The model under review builds one solid part; all positions refer to its coordinate system, in mm. Face numbers are marked on the shaded views. A direction names the side the tool comes from. Round coordinates to 2 decimals unless told otherwise and drop trailing zeros. Write each loop counter-clockwise with the first axis right and the second up, starting at its lowest first coordinate (ties: lowest second). Pieces come first, ordered by that corner, then holes. Notation, with made-up numbers: (24.25, 74) - (80.25, 74) arc R17 ccw to (80.25, 82) - close; hole circle Ø7 at (30, 88). An arc over 180 degrees is marked (long way). Write each question's results on one line, items separated by ' | '.
```python
from build123d import *

# Parameters (mm, degrees)
BOSS_EXTRUDE1_DEPTH   = 140
M8_TAPPED_HOLE1_D     = 6.8
M8_TAPPED_HOLE1_DEPTH = 19.75
M8_TAPPED_HOLE1_TIP   = 2.042926105


with BuildPart() as part:
    # Sketch1 → Boss-Extrude1 (new body)
    with BuildSketch(Plane.XY):
        with BuildLine():
            Line((0, 0), (0, 42.5))
            ThreePointArc((0, 42.5), (3.807611845, 51.692388155), (13, 55.5))
            Line((13, 55.5), (103, 55.5))
            ThreePointArc((103, 55.5), (112.192388155, 51.692388155), (116, 42.5))
            Line((116, 42.5), (116, 0))
            Line((116, 0), (108, 0))
            Line((108, 0), (108, 42.5))
            ThreePointArc((108, 42.5), (106.535533906, 46.035533906), (103, 47.5))
            Line((103, 47.5), (13, 47.5))
            ThreePointArc((13, 47.5), (9.464466094, 46.035533906), (8, 42.5))
            Line((8, 42.5), (8, 0))
            Line((8, 0), (0, 0))
        make_face()
    extrude(amount=BOSS_EXTRUDE1_DEPTH)

    # M8 Tapped Hole1
    with Locations(Plane(origin=(0, 55.5, 0), x_dir=(1, 0, 0), z_dir=(0, 1, 0))):
        with Locations((28.5, -13), (87.5, -13), (87.5, -53), (28.5, -53), (28.5, -87), (87.5, -87), (87.5, -127), (28.5, -127)):
            Hole(M8_TAPPED_HOLE1_D / 2, depth=M8_TAPPED_HOLE1_DEPTH)
            with Locations((0, 0, -(M8_TAPPED_HOLE1_DEPTH + M8_TAPPED_HOLE1_TIP / 2))):  # 118° drill point
                Cone(0, M8_TAPPED_HOLE1_D / 2, M8_TAPPED_HOLE1_TIP, mode=Mode.SUBTRACT)


solid = part.part
```
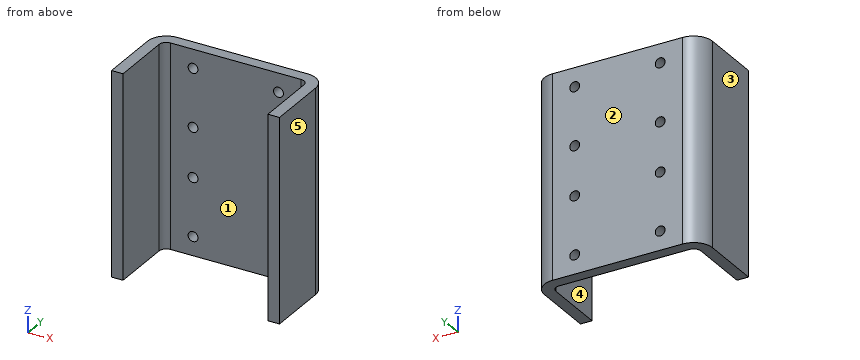
Q1. We need section D-D (y = 51.5). State how many separate pieces and enclosed holes the cut face has, plus the area to 3 significant figures.
Evaluation:
separate pieces: 1 | enclosed holes: 8 | area: 14,900 mm^2
Q2. Tool access review of the marked faces 4 and 5: name each direction out of +Z, -Z, +X, -X, +Y, -Y from which nothing blocks a thin tool from reaching the whole face with its end or side.
Evaluation:
face 4: +Z, -Z, -Y | face 5: +Z, -Z, +X, +Y, -Y
Q3. The part is to be moulded in two halves that separate along X. For the marked faces 1, 2 and 3, say which applies: released by +X, released by -X, zero draft, split by the parting line, or undercut.
Evaluation:
face 1: undercut | face 2: zero draft | face 3: released by -X
Q4. Insertion check: P1, Ø6, axis at x = 87.5, z = 53, coming from the -Y side; P2, Ø8, axis at x = 96, z = 65, coming from the -Y side. Each pin has a flat end and moves straight along its axis. Give the tip position at first contact, or say it passes through.
Evaluation:
P1: passes through | P2: stops at y = 47.5
Q5. We need section B-B (z = 13). State the section outline as (x, y) points, plus the area to 3 significant figures.
Evaluation:
outline: (0, 0) - (8, 0) - (8, 42.5) arc R5 cw to (13, 47.5) - (25.1, 47.5) - (25.1, 55.5) - (13, 55.5) arc R13 ccw to (0, 42.5) - close; (31.9, 47.5) - (84.1, 47.5) - (84.1, 55.5) - (31.9, 55.5) - close; (90.9, 47.5) - (103, 47.5) arc R5 cw to (108, 42.5) - (108, 0) - (116, 0) - (116, 42.5) arc R13 ccw to (103, 55.5) - (90.9, 55.5) - close | area: 1,520 mm^2
Q6. We need section A-A (y = 26). State the section outline as (x, z) points, plus the area to 3 significant figures.
Evaluation:
outline: (0, 0) - (8, 0) - (8, 140) - (0, 140) - close; (108, 0) - (116, 0) - (116, 140) - (108, 140) - close | area: 2,240 mm^2
Q7. We need section C-C (x = 28.5). State the section outline as (y, z) points, plus the area to 3 significant figures.
Evaluation:
outline: (47.5, 0) - (55.5, 0) - (55.5, 9.6) - (47.5, 9.6) - close; (47.5, 16.4) - (55.5, 16.4) - (55.5, 49.6) - (47.5, 49.6) - close; (47.5, 56.4) - (55.5, 56.4) - (55.5, 83.6) - (47.5, 83.6) - close; (47.5, 90.4) - (55.5, 90.4) - (55.5, 123.6) - (47.5, 123.6) - close; (47.5, 130.4) - (55.5, 130.4) - (55.5, 140) - (47.5, 140) - close | area: 902 mm^2
Q8. For probe 1 along Z at (x, y) = (87.5, 51.5); probe 2 along X at (y, z) = (53.25, 13); probe 3 along X at (y, z) = (9.5, 61), list the stretches that pass through material, from the lowest coordinate up.
Evaluation:
probe 1: z = 0 to 9.6, 16.4 to 49.6, 56.4 to 83.6, 90.4 to 123.6, 130.4 to 140 | probe 2: x = 5.69 to 25.1, 31.9 to 84.1, 90.9 to 110.31 | probe 3: x = 0 to 8, 108 to 116
